```python
from build123d import *

# Parameters (mm, degrees)
SKETCH_1_W          = 200.4
SKETCH_1_H          = 146.5
EXTRUDE_1_DEPTH     = 17
SKETCH_2_W          = 175
SKETCH_2_H          = 120
CUT_EXTRUDE_1_DEPTH = 0.5
SKETCH_3_W          = 200.4
SKETCH_3_H          = 146.5
SKETCH_3_W_2        = 190
SKETCH_3_H_2        = 136
CUT_EXTRUDE_2_DEPTH = 30
FILLET_1_R          = 3
SKETCH_4_W          = 40
SKETCH_4_H          = 8
EXTRUDE_2_DEPTH     = 40
SKETCH_5_W          = 15
SKETCH_5_H          = 8
EXTRUDE_3_DEPTH     = 20
FILLET_2_R          = 2
SKETCH_6_R          = 1.75
EXTRUDE_4_DEPTH     = 5
CUT_EXTRUDE_3_DEPTH = 151.973640083
SKETCH_8_W          = 5
SKETCH_8_H          = 15
CUT_EXTRUDE_4_DEPTH = 151.973640083
SKETCH_9_R          = 1.5
EXTRUDE_5_DEPTH     = 35


with BuildPart() as part:
    # 草图1 → 凸台-拉伸1 (new, symmetric)
    with BuildSketch(Plane(origin=(0, 0, 0), x_dir=(1, 0, 0), z_dir=(0, 1, 0))):
        Rectangle(SKETCH_1_W, SKETCH_1_H)
    extrude(amount=EXTRUDE_1_DEPTH, both=True)

    # 草图2 → 切除-拉伸1 (cut)
    with BuildSketch(Plane(origin=(0, 17, 0), x_dir=(1, 0, 0), z_dir=(0, 1, 0))):
        Rectangle(SKETCH_2_W, SKETCH_2_H)
    extrude(amount=-CUT_EXTRUDE_1_DEPTH, mode=Mode.SUBTRACT)

    # 草图3 → 切除-拉伸2 (cut)
    with BuildSketch(Plane.XZ.offset(17)):
        Rectangle(SKETCH_3_W, SKETCH_3_H)
        Rectangle(SKETCH_3_W_2, SKETCH_3_H_2, mode=Mode.SUBTRACT)
    extrude(amount=-CUT_EXTRUDE_2_DEPTH, mode=Mode.SUBTRACT)

    # 圆角1
    fillet_1_edges = [part.edges().sort_by_distance(p)[0] for p in [
        (-100.2, 15, -73.25),
        (100.2, 15, -73.25),
        (100.2, 15, 73.25),
        (-100.2, 15, 73.25),
    ]]
    fillet(fillet_1_edges, radius=FILLET_1_R)

    # 草图4 → 凸台-拉伸2 (add)
    with BuildSketch(Plane(origin=(0, 0, -68), x_dir=(-1, 0, 0), z_dir=(0, 0, -1))):
        with Locations((9.8, -12)):
            Rectangle(SKETCH_4_W, SKETCH_4_H)
    extrude(amount=EXTRUDE_2_DEPTH)

    # 草图5 → 凸台-拉伸3 (add)
    with BuildSketch(Plane(origin=(0, 0, -68), x_dir=(-1, 0, 0), z_dir=(0, 0, -1))):
        with Locations((-72.7, -9)):
            Rectangle(SKETCH_5_W, SKETCH_5_H)
    extrude(amount=EXTRUDE_3_DEPTH)

    # 圆角2
    fillet_2_edges = [part.edges().sort_by_distance(p)[0] for p in [
        (65.2, -13, -78),
        (65.2, -5, -78),
        (80.2, -5, -78),
        (80.2, -13, -78),
        (65.2, -9, -88),
        (72.7, -5, -88),
        (80.2, -9, -88),
        (72.7, -13, -88),
    ]]
    fillet(fillet_2_edges, radius=FILLET_2_R)

    # 草图6 → 凸台-拉伸4 (add)
    with BuildSketch(Plane(origin=(0, 0, -88), x_dir=(-1, 0, 0), z_dir=(0, 0, -1))):
        with Locations((-72.7, -9)):
            Circle(SKETCH_6_R)
    extrude(amount=EXTRUDE_4_DEPTH)

    # 草图7 → 切除-拉伸3 (cut, through all)
    with BuildSketch(Plane.XZ.offset(16)):
        Polygon((-29.8, -88), (-19.8, -88), (-14.8, -98), (-14.8, -108), (-29.8, -108), align=None)
        Polygon((-4.8, -98), (-4.8, -108), (10.2, -108), (10.2, -88), (0.2, -88), align=None)
    extrude(amount=-CUT_EXTRUDE_3_DEPTH, mode=Mode.SUBTRACT)

    # 草图8 → 切除-拉伸4 (cut, through all)
    with BuildSketch(Plane.XZ.offset(16)):
        with Locations((-27.3, -80.5)):
            Rectangle(SKETCH_8_W, SKETCH_8_H)
        with Locations((7.7, -80.5)):
            Rectangle(SKETCH_8_W, SKETCH_8_H)
    extrude(amount=-CUT_EXTRUDE_4_DEPTH, mode=Mode.SUBTRACT)

    # 草图9 → 凸台-拉伸5 (add)
    with BuildSketch(Plane(origin=(0, 0, -73), x_dir=(-1, 0, 0), z_dir=(0, 0, -1))):
        with Locations(Location((27.3, -12, 0), (0, 0, 270))):
            Circle(SKETCH_9_R)
        with Locations(Location((-7.7, -12, 0), (0, 0, 270))):
            Circle(SKETCH_9_R)
    extrude(amount=EXTRUDE_5_DEPTH)


solid = part.part
```
Could you check a few things on this model? Use its own coordinates, in mm. A direction names the side the tool comes from. Round coordinates to 2 decimals unless told otherwise and drop trailing zeros. Loops run counter-clockwise (first coordinate to the right, second up) from the corner with the lowest first, then second, coordinate; pieces in that order, holes last. Notation, with made-up numbers: M 88.5,77.5 L 97.5,77.5 A20 ccw 97.5,107.5 Z; hole C 69,42 d6. An arc over 180 degrees is marked long. Put each result on its own line as item: value.
Q1. Imagine slicing it at D-D (y = -1). Write out the boundary of the cut face in (x, z), then the cut area to 3 significant figures.
Check result:
outline: M -95,-68 L 95,-68 L 95,68 L -95,68 Z
area: 25,800 mm2
Q2. Imagine slicing it at C-C (z = -7). Write out the boundary of the cut face in (x, y).
Check result:
outline: M -100.2,13 L -95,13 L -95,-17 L 95,-17 L 95,13 L 100.2,13 L 100.2,17 L 87.5,17 L 87.5,16.5 L -87.5,16.5 L -87.5,17 L -100.2,17 Z
Q3. For pin 1 (4 mm diameter, centred on x = -21.5, y = -11, fed in from -Z); pin 2 (1.2 mm diameter, centred on x = -15, y = 15.5, fed in from -Z); pin 3 (12 mm diameter, centred on y = 5.5, z = -40.5, fed in from -X), each with a flat end and sliding along its axis, tell me the tip position at first contact or that it passes through.
Check result:
pin 1: z = -88.6
pin 2: z = -73.25
pin 3: x = -95
Q4. Thinking about a two-plate mould opening in Y: for faces 1 (the face through (73, -5, -77)), 2 (the face through (-10, -16, -83)), 3 (the face through (-10, -8, -83)), 4 (the face through (-2.265, -12.056, -92.93)), which applies, released by +Y, released by -Y, zero draft, split by the parting line, or undercut?
Check result:
face 1: undercut
face 2: released by -Y
face 3: undercut
face 4: zero draft
Q5. On a 3-axis mill with a long thin cutter (end or side, diameter ignored), from which of +Z, -Z, +X, -X, +Y, -Y can I reach the whole of each face in a straight line? I mean faces 5 (the face through (3, -12, -88)), 6 (the face through (73, -13, -77)), 7 (the face through (6, -12, -73)). Say none if no direction works.
Check result:
face 5: -Z, +Y, -Y
face 6: -Z, +X, -Y
face 7: -Z
Q6. Imagine slicing it at A-A (z = -79.5). Write out the boundary of the cut face in (x, y).
Check result:
outline: C -27.3,-12 d3; M -24.8,-16 L 5.2,-16 L 5.2,-8 L -24.8,-8 Z; C 7.7,-12 d3; M 65.2,-11 A2 ccw 67.2,-13 L 78.2,-13 A2 ccw 80.2,-11 L 80.2,-7 A2 ccw 78.2,-5 L 67.2,-5 A2 ccw 65.2,-7 Z
Q7. I need wall thicknesses on probe 1 along X at (y, z) = (-7.5, 47); probe 2 along Z at (x, y) = (1, 6.5); probe 3 along Y at (x, z) = (24, 49). Which ranges of each line are inside material? Lowest first, please.
Check result:
probe 1: -95 to 95
probe 2: -68 to 68
probe 3: -17 to 16.5
Q8. Imagine slicing it at B-B (x = -11.5). Write out the boundary of the cut face in (y, z), then the cut area to 3 significant figures.
Check result:
outline: M -17,-68 L -16,-68 L -16,-108 L -8,-108 L -8,-68 L 13,-68 L 13,-73.25 L 17,-73.25 L 17,-60 L 16.5,-60 L 16.5,60 L 17,60 L 17,73.25 L 13,73.25 L 13,68 L -17,68 Z
area: 4,930 mm2
